from build123d import *
from build123d.topology import SkipClean

# Parameters (mm, degrees)
BASE_PLATE_PROFILE_W   = 12
BASE_PLATE_PROFILE_H   = 23
BASE_PLATE_DEPTH       = 10
GROOVE_PROFILE_4X5_W   = 4
GROOVE_PROFILE_4X5_H   = 5
GROOVE_CUT_4X5_DEPTH   = 150
ARM_DEPTH              = 12
EYE_START              = 5
EYE_BOSS_SKETCH_30_R   = 15
EYE_BOSS_30_DEPTH      = 5
ARM_START              = -4
ARM_RELIEF_CUT_DEPTH   = 4
EYE_HOLE_SKETCH_12_R   = 6
EYE_HOLE_12_DEPTH      = 20
UPRIGHT_RIB_DEPTH      = 8
CROSS_HOLE_SKETCH_12_R = 6
CROSS_HOLE_12_DEPTH    = 20
UPRIGHT_WEB_DEPTH      = 72
WEB_TRIM_CUT_1_DEPTH   = 31
WEB_TRIM_CUT_2_DEPTH   = 31


with BuildPart() as part:
    # Base Plate Profile → Base Plate (new body)
    with BuildSketch(Plane.XY):
        Polygon((36, 0), (12, 0), (12, -23), (60, -23), (60, 0), align=None)
        with Locations((6, -11.5)):
            Rectangle(BASE_PLATE_PROFILE_W, BASE_PLATE_PROFILE_H)
        with Locations((66, -11.5)):
            Rectangle(BASE_PLATE_PROFILE_W, BASE_PLATE_PROFILE_H)
        with BuildLine():
            Line((12, -35), (60, -35))
            ThreePointArc((60, -35), (68.485281374, -31.485281374), (72, -23))
            Line((72, -23), (0, -23))
            ThreePointArc((0, -23), (3.514718626, -31.485281374), (12, -35))
        make_face()
    extrude(amount=BASE_PLATE_DEPTH)

    # Groove Profile 4x5 → Groove Cut 4x5 (cut)
    with BuildSketch(Plane(origin=(72, 0, 0), x_dir=(0, 0, -1), z_dir=(1, 0, 0))):
        with Locations((-8, -2.5)):
            Rectangle(GROOVE_PROFILE_4X5_W, GROOVE_PROFILE_4X5_H)
    extrude(amount=-GROOVE_CUT_4X5_DEPTH, mode=Mode.SUBTRACT)

    # Arm Profile → Arm (add)
    with BuildSketch(Plane(origin=(0, -5, 0), x_dir=(1, 0, 0), z_dir=(0, 1, 0))):
        with BuildLine():
            Line((21, -60), (21, -10))
            Line((21, -10), (51, -10))
            Line((51, -10), (51, -60))
            ThreePointArc((51, -60), (36, -75), (21, -60))
        make_face()
    extrude(amount=-ARM_DEPTH)

    # Eye Boss Sketch Ø30 → Eye Boss Ø30 (add)
    with SkipClean():  # the faces are left unmerged after this step: merging them gives an invalid solid
        with BuildSketch(Plane(origin=(0, -5, 0), x_dir=(1, 0, 0), z_dir=(0, 1, 0)).offset(EYE_START)):
            with Locations(Location((36, -60, 0), (0, 0, 180))):
                Circle(EYE_BOSS_SKETCH_30_R)
        extrude(amount=-EYE_BOSS_30_DEPTH)

    # Arm Relief Profile → Arm Relief Cut (cut)
    with SkipClean():  # the faces are left unmerged after this step: merging them gives an invalid solid
        with BuildSketch(Plane.XZ.offset(17).offset(ARM_START)):
            with BuildLine():
                Line((21, 10), (21, 60))
                ThreePointArc((21, 60), (36, 75), (51, 60))
                Line((51, 60), (51, 10))
                Line((51, 10), (21, 10))
            make_face()
        extrude(amount=ARM_RELIEF_CUT_DEPTH, mode=Mode.SUBTRACT)

    # Eye Hole Sketch Ø12 → Eye Hole Ø12 (cut)
    with SkipClean():  # the faces are left unmerged after this step: merging them gives an invalid solid
        with BuildSketch(Plane.XZ.offset(13)):
            with Locations((36, 60)):
                Circle(EYE_HOLE_SKETCH_12_R)
        extrude(amount=-EYE_HOLE_12_DEPTH, mode=Mode.SUBTRACT)

    # Upright Rib Profile → Upright Rib (add)
    with SkipClean():  # the faces are left unmerged after this step: merging them gives an invalid solid
        with BuildSketch(Plane.XZ.offset(13)):
            with BuildLine():
                Line((6, 10), (21, 10))
                Line((21, 10), (21, 25))
                ThreePointArc((21, 25), (16.606601718, 14.393398282), (6, 10))
            make_face()
            with BuildLine():
                Line((51, 25), (51, 10))
                Line((51, 10), (66, 10))
                ThreePointArc((66, 10), (55.393398282, 14.393398282), (51, 25))
            make_face()
        extrude(amount=-UPRIGHT_RIB_DEPTH)

    # Cross Hole Sketch Ø12 → Cross Hole Ø12 (cut)
    with SkipClean():  # the faces are left unmerged after this step: merging them gives an invalid solid
        with BuildSketch(Plane.XY.offset(10)):
            with Locations((12, -23)):
                Circle(CROSS_HOLE_SKETCH_12_R)
            with Locations((60, -23)):
                Circle(CROSS_HOLE_SKETCH_12_R)
        extrude(amount=-CROSS_HOLE_12_DEPTH, mode=Mode.SUBTRACT)

    # Upright Web Profile → Upright Web (add)
    with SkipClean():  # the faces are left unmerged after this step: merging them gives an invalid solid
        with BuildSketch(Plane.ZY):
            Polygon((10, -13), (45.07175112, -13), (10, -35), align=None)
        extrude(amount=-UPRIGHT_WEB_DEPTH)

    # Web Trim Profile 1 → Web Trim Cut 1 (cut)
    with SkipClean():  # the faces are left unmerged after this step: merging them gives an invalid solid
        with BuildSketch(Plane(origin=(72, 0, 0), x_dir=(0, 0, -1), z_dir=(1, 0, 0))):
            Polygon((-45.07175112, -13), (-10, -13), (-10, -35), align=None)
        extrude(amount=-WEB_TRIM_CUT_1_DEPTH, mode=Mode.SUBTRACT)

    # Web Trim Profile 2 → Web Trim Cut 2 (cut)
    with SkipClean():  # the faces are left unmerged after this step: merging them gives an invalid solid
        with BuildSketch(Plane.ZY):
            Polygon((10, -35), (10, -13), (45.07175112, -13), align=None)
        extrude(amount=-WEB_TRIM_CUT_2_DEPTH, mode=Mode.SUBTRACT)


solid = part.part
Source: CAD feature listing. Evaluate the final solid. Frame: model axes, mm. A direction names the side the tool comes from. Give positions to 0.01 mm unless a question says otherwise; leave off trailing zeros. Write each loop counter-clockwise with the first axis right and the second up, starting at its lowest first coordinate (ties: lowest second). Pieces come first, ordered by that corner, then holes. Notation, with made-up numbers: (15.5, -18.75) - (56.5, -18.75) arc R12 ccw to (56.5, -2.75) - close; hole circle Ø8 at (2.25, 53.25). An arc over 180 degrees is marked (long way). Write item = value, one per line. Start each with the question number.
Q1. Cut plane C-C, the plane z = 20. Return loops of the section in (x, y), then the cut area to 3 significant figures.
Q2. Draft query along X for faces 5 (the cylindrical face through (17.54, -25.3, 5.07)), 6 (the flat face through (35, -17, 0)), 7 (the flat face through (0, -12, 5)), 8 (the cylindrical face through (54, -23, 5)). Return one class per face: +X half, -X half, draft (parallel to the pull), parting line (faces both ways), or undercut.
Q3. Cut plane D-D, the plane x = 45.5. Return loops of the section in (y, z).
Q4. Cut plane A-A, the plane x = 36. Return loops of the section in (y, z).
Q5. Reachability of faces 1 (the flat face through (51, -9, 42)), 2 (the flat face through (37, -3, 6)), 3 (the flat face through (41, -21, 23)), 4 (the flat face through (42, -13, 42)) from +Z, -Z, +X, -X, +Y, -Y: full face, straight path, thin tool, end or side. Return the list, or none.
Q6. Pin query (flat end, axial travel): pin 1 Ø10 at (x, y) = (56, -19) entering from +Z; pin 2 Ø16 at (x, z) = (32.5, 46.5) entering from +Y; pin 3 Ø5 at (y, z) = (-8, 23.5) entering from +X; pin 4 Ø9 at (y, z) = (-8.5, 41.5) entering from -X. Return the tip coordinate at first contact, or that it passes through.
Q7. Material intervals for probe 1 along Y at (x, z) = (60, 5.25); probe 2 along Y at (x, z) = (42, 28); probe 3 along X at (y, z) = (-25, 16), sorted ascending.
Q8. Cut plane B-B, the plane z = 55.5. Return loops of the section in (x, y).
Computed values:
q1.outline = (20.14, -13) - (31, -13) - (31, -28.73) - (41, -28.73) - (41, -13) - (51.86, -13) - (51.86, -5) - (20.14, -5) - close
q1.area = 411 mm²
q2.face_5 = undercut
q2.face_6 = draft
q2.face_7 = -X half
q2.face_8 = undercut
q3.outline = (-35, 0) - (0, 0) - (0, 6) - (-5, 6) - (-5, 48.39) - (0, 48.39) - (0, 71.61) - (-13, 71.61) - (-13, 10) - (-35, 10) - close
q4.outline = (-35, 0) - (0, 0) - (0, 6) - (-5, 6) - (-5, 45) - (0, 45) - (0, 54) - (-13, 54) - (-13, 45.07) - (-35, 10) - close; (-13, 66) - (0, 66) - (0, 75) - (-13, 75) - close
q5.face_1 = +Z, +X, +Y, -Y
q5.face_2 = +X, -X, +Y
q5.face_3 = +Z, +X, -Y
q5.face_4 = +Z, -Y
q6.pin_1 = 10
q6.pin_2 = 0
q6.pin_3 = 51.54
q6.pin_4 = 21
q7.probe_1 = -35 to -29, -17 to 0
q7.probe_2 = -13 to -5
q7.probe_3 = 31 to 41
q8.outline = (21, -13) - (32.03, -13) - (32.03, 0) - (21.69, 0) - (21.69, -5) - (21, -5) - close; (39.97, -13) - (51, -13) - (51, -5) - (50.31, -5) - (50.31, 0) - (39.97, 0) - close
